from build123d import *

# Parameters (mm, degrees)
BOSS_EXTRUDE1_DEPTH = 5
SKETCH2_W           = 30
SKETCH2_H           = 200
CUT_EXTRUDE1_DEPTH  = 10


with BuildPart() as part:
    # Sketch1 → Boss-Extrude1 (new, symmetric)
    with BuildSketch(Plane.XY):
        with BuildLine():
            Line((-63.274211694, 196.041766301), (-20, 40))
            Line((-20, 40), (-20, 30))
            Line((-20, 30), (20, 30))
            Line((20, 30), (20, 40))
            Line((20, 40), (63.274211694, 196.041766301))
            ThreePointArc((63.274211694, 196.041766301), (0, 206), (-63.274211694, 196.041766301))
        make_face()
    extrude(amount=BOSS_EXTRUDE1_DEPTH, both=True)

    # Sketch2 → Cut-Extrude1 (cut)
    with BuildSketch(Plane.XY.offset(5)):
        with Locations((0, 30)):
            Rectangle(SKETCH2_W, SKETCH2_H)
    extrude(amount=-CUT_EXTRUDE1_DEPTH, mode=Mode.SUBTRACT)


solid = part.part
Can you work these out from the model? Positions are in its coordinate system, mm. A direction names the side the tool comes from. Coordinates: 2 decimals unless noted, no trailing zeros. Order: outer loops, then holes, each group sorted by start corner. A loop starts at its lowest first (then second) coordinate and runs counter-clockwise, first axis right, second up. Notation, with made-up numbers: (61, 58) - (98, 58) arc R10 cw to (98, 67) - close; hole circle Ø7 at (-24, 2). An arc over 180 degrees is marked (long way). Answer as a JSON object with one key per item and string values. Group by question number.
Q1. Imagine slicing it at A-A (y = 106). Please give me the cut outline in (x, z).
Q2. I need wall thicknesses on line 1 (X direction, y = 37, z = -1.25); line 2 (X direction, y = 43, z = -2); line 3 (Y direction, x = 0, z = -4). Which ranges of each line are inside material? Lowest first, please. Write a range as from..to.
Q3. Imagine slicing it at D-D (y = 192.5). Please give me the cut outline in (x, z), and give its area (3 significant figures).
Q4. On a 3-axis mill with a long thin cutter (end or side, diameter ignored), from which of +Z, -Z, +X, -X, +Y, -Y can I reach the whole of each face in a straight line? I mean faces 1 (the face through (20, 35, 0)), 2 (the face through (-20, 35, 0)), 3 (the face through (15, 79, 0)). Say none if no direction works.
Q5. Will these pins go through, and if not, where does the flat tip stop? P1, Ø1.5, axis at y = 50.5, z = -3.5, coming from the -X side; P2, Ø5, axis at x = 0, z = -1, coming from the -Y side; P3, Ø3, axis at y = 36, z = -1.5, coming from the -X side.
Q6. Imagine slicing it at C-C (x = 10). Please give me the cut outline in (y, z).
Q7. Imagine slicing it at B-B (z = -0.25). Please give me the cut outline in (x, y), and give its area (3 significant figures).
Determined:
{
 "1": {"outline": "(-38.3, -5) - (-15, -5) - (-15, 5) - (-38.3, 5) - close; (15, -5) - (38.3, -5) - (38.3, 5) - (15, 5) - close"},
 "2": {"line 1": "x = -20..-15, 15..20", "line 2": "x = -20.83..-15, 15..20.83", "line 3": "y = 130..206"},
 "3": {"outline": "(-62.29, -5) - (62.29, -5) - (62.29, 5) - (-62.29, 5) - close", "area": "1,250 mm2"},
 "4": {"face 1": "+Z, -Z, +X, -Y", "face 2": "+Z, -Z, -X, -Y", "face 3": "+Z, -Z, -Y"},
 "5": {"P1": "stops at x = -23.12", "P2": "stops at y = 130", "P3": "stops at x = -20"},
 "6": {"outline": "(130, -5) - (205.76, -5) - (205.76, 5) - (130, 5) - close"},
 "7": {"outline": "(-63.27, 196.04) - (-20, 40) - (-20, 30) - (-15, 30) - (-15, 130) - (15, 130) - (15, 30) - (20, 30) - (20, 40) - (63.27, 196.04) arc R206 ccw to start", "area": "11,200 mm2"}
}
